```python
from build123d import *

# Parameters (mm, degrees)
SKETCH1_R           = 12.1
SKETCH1_R_2         = 65
SKETCH1_R_3         = 30.1
BOSS_EXTRUDE1_DEPTH = 3


with BuildPart() as part:
    # Sketch1 → Boss-Extrude1 (new body)
    with BuildSketch(Plane.XY):
        with BuildLine():
            Line((2, 0), (548, 0))
            ThreePointArc((548, 0), (549.414213562, 0.585786438), (550, 2))
            Line((550, 2), (550, 708))
            ThreePointArc((550, 708), (549.414213562, 709.414213562), (548, 710))
            Line((548, 710), (2, 710))
            ThreePointArc((2, 710), (0.585786438, 709.414213562), (0, 708))
            Line((0, 708), (0, 2))
            ThreePointArc((0, 2), (0.585786438, 0.585786438), (2, 0))
        make_face()
        with Locations((40, 60)):
            Circle(SKETCH1_R, mode=Mode.SUBTRACT)
        with Locations((40, 120)):
            Circle(SKETCH1_R, mode=Mode.SUBTRACT)
        with Locations((40, 180)):
            Circle(SKETCH1_R, mode=Mode.SUBTRACT)
        with Locations((430, 110)):
            Circle(SKETCH1_R_2, mode=Mode.SUBTRACT)
        with Locations((310, 605)):
            Circle(SKETCH1_R_3, mode=Mode.SUBTRACT)
    extrude(amount=BOSS_EXTRUDE1_DEPTH)


solid = part.part
```
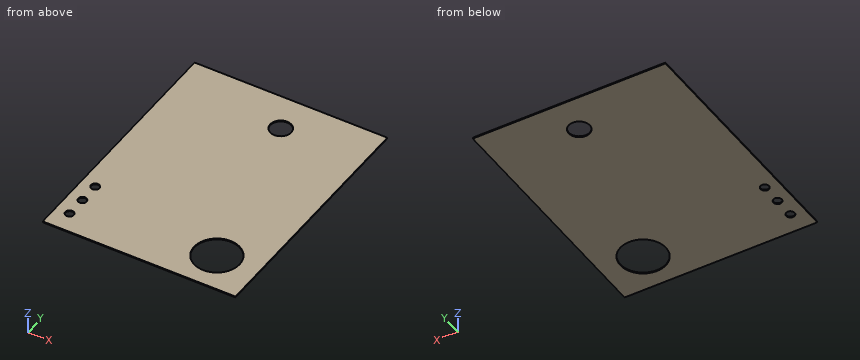
Input: part model. Units: mm. Frame: model coordinates. Round coordinates to 2 decimals unless told otherwise and drop trailing zeros. Loops run counter-clockwise (first coordinate to the right, second up) from the corner with the lowest first, then second, coordinate; pieces in that order, holes last. Notation, with made-up numbers: (58, 61) -> (66, 61) arc R13 cw to (66, 71) -> close; hole circle Ø10 at (10, 85). An arc over 180 degrees is marked (long way). Use one line per item in the form item = value. Start each with the question number.
Item 1: Section query A-A on x = 430. Return the cut outline in (y, z), then the cut area to 3 significant figures.
Item 2: Section query D-D on y = 605. Return the cut outline in (x, z), then the cut area to 3 significant figures.
Item 3: Section query C-C on x = 40. Return the cut outline in (y, z).
Item 4: Contact query for a flat-ended pin moving along its axis: pin 1 Ø12 at (x, y) = (123, 348.5) entering from -Z. Output: stop coordinate, or through.
Item 5: Section query B-B on z = 2.35. Return the cut outline in (x, y).
Item 6: Material intervals for L1, parallel to Y at x = 40, z = 1.4; L2, parallel to Y at x = 310, z = 2.3; L3, parallel to Y at x = 432, z = 1.2, sorted ascending. Write a range as from..to.
Ans:
q1.outline = (0, 0) -> (45, 0) -> (45, 3) -> (0, 3) -> close; (175, 0) -> (710, 0) -> (710, 3) -> (175, 3) -> close
q1.area = 1,740 mm^2
q2.outline = (0, 0) -> (279.9, 0) -> (279.9, 3) -> (0, 3) -> close; (340.1, 0) -> (550, 0) -> (550, 3) -> (340.1, 3) -> close
q2.area = 1,470 mm^2
q3.outline = (0, 0) -> (47.9, 0) -> (47.9, 3) -> (0, 3) -> close; (72.1, 0) -> (107.9, 0) -> (107.9, 3) -> (72.1, 3) -> close; (132.1, 0) -> (167.9, 0) -> (167.9, 3) -> (132.1, 3) -> close; (192.1, 0) -> (710, 0) -> (710, 3) -> (192.1, 3) -> close
q4.pin_1 = 0
q5.outline = (0, 2) arc R2 ccw to (2, 0) -> (548, 0) arc R2 ccw to (550, 2) -> (550, 708) arc R2 ccw to (548, 710) -> (2, 710) arc R2 ccw to (0, 708) -> close; hole circle Ø24.2 at (40, 60); hole circle Ø24.2 at (40, 120); hole circle Ø24.2 at (40, 180); hole circle Ø60.2 at (310, 605); hole circle Ø130 at (430, 110)
q6.L1 = 0..47.9, 72.1..107.9, 132.1..167.9, 192.1..710
q6.L2 = 0..574.9, 635.1..710
q6.L3 = 0..45.03, 174.97..710
